Could you check a few things on this model? Use its own coordinates, in mm. A direction names the side the tool comes from. Coordinates: 2 decimals unless noted, no trailing zeros. Loops run counter-clockwise (first coordinate to the right, second up) from the corner with the lowest first, then second, coordinate; pieces in that order, holes last.
from build123d import *

# Parameters (mm, degrees)
EXTRUDE_1_DEPTH     = 1500
SKETCH_2_R          = 2.75
CUT_EXTRUDE_1_DEPTH = 10


with BuildPart() as part:
    # 草图1 → 拉伸-薄壁1 (new body)
    with BuildSketch(Plane.XY):
        Polygon((54, 5), (54, 0), (0, 0), (0, -15), (-1.5, -15), (-1.5, 1.5), (52.5, 1.5), (52.5, 5), align=None)
    extrude(amount=EXTRUDE_1_DEPTH)

    # 草图2 → 切除-拉伸1 (cut)
    with BuildSketch(Plane(origin=(0, 0, 0), x_dir=(0, 0, -1), z_dir=(1, 0, 0))):
        with Locations(Location((-1450, -7.5, 0), (0, 0, 90))):
            Circle(SKETCH_2_R)
        with Locations(Location((-1100, -7.5, 0), (0, 0, 90))):
            Circle(SKETCH_2_R)
        with Locations(Location((-750, -7.5, 0), (0, 0, 90))):
            Circle(SKETCH_2_R)
        with Locations(Location((-400, -7.5, 0), (0, 0, 90))):
            Circle(SKETCH_2_R)
        with Locations(Location((-50, -7.5, 0), (0, 0, 90))):
            Circle(SKETCH_2_R)
    extrude(amount=-CUT_EXTRUDE_1_DEPTH, mode=Mode.SUBTRACT)


solid = part.part
(1) Imagine slicing it at A-A, the plane z = 654.5. Write out the boundary of the cut face in (x, y), and give its area (3 significant figures).
Answers:
outline: (-1.5, -15) - (0, -15) - (0, 0) - (54, 0) - (54, 5) - (52.5, 5) - (52.5, 1.5) - (-1.5, 1.5) - close
area: 111 mm2
(2) Which directions (+Z, -Z, +X, -X, +Y, -Y) give clear straight access to the entire face, cutting with the end or side of a thin tool? Please do faces 1 (the face through (27, 0, 740)), 2 (the face through (25, 1.5, 740)).
Answers:
face 1: +Z, -Z, +X, -Y
face 2: +Z, -Z, -X, +Y
(3) I need wall thicknesses on probe 1 along Z at (x, y) = (-1.05, -7.5); probe 2 along Y at (x, z) = (14.5, 220.5); probe 3 along X at (y, z) = (-4, 1197.5). Which ranges of each line are inside material? Lowest first, please.
Answers:
probe 1: z = 0 to 47.25, 52.75 to 397.25, 402.75 to 747.25, 752.75 to 1097.25, 1102.75 to 1447.25, 1452.75 to 1500
probe 2: y = 0 to 1.5
probe 3: x = -1.5 to 0
(4) For pin 1 (3 mm diameter, centred on y = 3.5, z = 1059.5, fed in from -X); pin 2 (9 mm diameter, centred on y = -7.5, z = 400, fed in from +X); pin 3 (1.5 mm diameter, centred on x = 43.5, z = 300.5, fed in from +Y); pin 4 (6 mm diameter, centred on x = 40, y = -3.5, fed in from +Z), each with a flat end and sliding along its axis, tell me the tip position at first contact or that it passes through.
Answers:
pin 1: stops at x = 52.5
pin 2: stops at x = 0
pin 3: stops at y = 1.5
pin 4: passes through
(5) Imagine slicing it at B-B, the plane x = 31.5. Write out the boundary of the cut face in (y, z), and give its area (3 significant figures).
Answers:
outline: (0, 0) - (1.5, 0) - (1.5, 1500) - (0, 1500) - close
area: 2,250 mm2
